from build123d import *

# Parameters (mm, degrees)
SKETCH_1_W             = 80
SKETCH_1_H             = 98.4
EXTRUDE_1_DEPTH        = 14
HOLE_WIZARD_M6_1_D     = 5
HOLE_WIZARD_M6_1_DEPTH = 17
HOLE_WIZARD_M6_1_TIP   = 1.502151548
HOLE_WIZARD_M6_2_D     = 5
HOLE_WIZARD_M6_2_DEPTH = 17
HOLE_WIZARD_M6_2_TIP   = 1.502151548


with BuildPart() as part:
    # 草图1 → 凸台-拉伸1 (new body)
    with BuildSketch(Plane.XY):
        Rectangle(SKETCH_1_W, SKETCH_1_H)
    extrude(amount=EXTRUDE_1_DEPTH)

    # M6 螺纹孔1
    with Locations(Plane(origin=(0, -49.2, 0), x_dir=(-1, 0, 0), z_dir=(0, -1, 0))):
        with Locations((-21, -7), (21, -7)):
            Hole(HOLE_WIZARD_M6_1_D / 2, depth=HOLE_WIZARD_M6_1_DEPTH)
            with Locations((0, 0, -(HOLE_WIZARD_M6_1_DEPTH + HOLE_WIZARD_M6_1_TIP / 2))):  # 118° drill point
                Cone(0, HOLE_WIZARD_M6_1_D / 2, HOLE_WIZARD_M6_1_TIP, mode=Mode.SUBTRACT)

    # M6 螺纹孔2
    with Locations(Plane(origin=(0, 49.2, 0), x_dir=(1, 0, 0), z_dir=(0, 1, 0))):
        with Locations((-17.5, -7), (17.5, -7)):
            Hole(HOLE_WIZARD_M6_2_D / 2, depth=HOLE_WIZARD_M6_2_DEPTH)
            with Locations((0, 0, -(HOLE_WIZARD_M6_2_DEPTH + HOLE_WIZARD_M6_2_TIP / 2))):  # 118° drill point
                Cone(0, HOLE_WIZARD_M6_2_D / 2, HOLE_WIZARD_M6_2_TIP, mode=Mode.SUBTRACT)


solid = part.part
Geometry check sheet. Reference: the model listing, model coordinates, mm. A direction names the side the tool comes from. Round coordinates to 2 decimals unless told otherwise and drop trailing zeros. Order: outer loops, then holes, each group sorted by start corner. A loop starts at its lowest first (then second) coordinate and runs counter-clockwise, first axis right, second up. Notation, with made-up numbers: (-16.5, 10.25) -> (12.5, 10.25) arc R13 ccw to (12.5, 19.25) -> close; hole circle Ø1 at (68.5, 66). An arc over 180 degrees is marked (long way). Use one line per item in the form item = value.
1. Scan lines: line 1 along Z through (x, y) = (17.5, 42.5); line 2 along Z through (x, y) = (17, 43). Record each from-to range of solid material in increasing order. Write a range as from..to.
Working result:
line_1 = 0..4.5, 9.5..14
line_2 = 0..4.55, 9.45..14
2. Cross-section at A-A, the plane y = -37.5. Enter the section's corners in (x, z), plus the area to 3 significant figures.
Working result:
outline = (-40, 0) -> (40, 0) -> (40, 14) -> (-40, 14) -> close; hole circle Ø5 at (-21, 7); hole circle Ø5 at (21, 7)
area = 1,080 mm^2
3. Go/stop test with flat-tipped pins: pin 1 (1.5 mm diameter, centred on x = 14, y = -5.5, fed in from -Z); pin 2 (4 mm diameter, centred on x = 21, z = 7, fed in from -Y); pin 3 (4.5 mm diameter, centred on x = -21, z = 7, fed in from -Y); pin 4 (4.5 mm diameter, centred on x = -17.5, z = 7, fed in from +Y). Record where each tip stops, or that it passes through.
Working result:
pin_1 = 0
pin_2 = -31.9
pin_3 = -32.05
pin_4 = 32.05
4. Mould release check, pull along X, two halves, no side actions. Record for faces 4 (the face through (-40, -1, 7)), 5 (the face through (40, -1, 7)), 6 (the face through (-1, 1, 0)), 7 (the face through (17, 31, 7)): pulls with the +X half, pulls with the -X half, needs draft (parallel to the pull), parting line crosses it, or undercut.
Working result:
face_4 = pulls with the -X half
face_5 = pulls with the +X half
face_6 = needs draft
face_7 = undercut
5. Set-up check for faces 1 (the face through (18.5, -40.6, 6.9)), 2 (the face through (-1, 1, 14)), 3 (the face through (20, 41, 7)): record each of +Z, -Z, +X, -X, +Y, -Y from which the full face is reachable in a straight line by a thin tool's end or side.
Working result:
face_1 = -Y
face_2 = +Z, +X, -X, +Y, -Y
face_3 = +Y
